Read the model definition and answer for the solid it produces. Units are mm, in the model's axes. Face numbers are marked on the shaded views. Round coordinates to 2 decimals unless told otherwise and drop trailing zeros. Order: outer loops, then holes, each group sorted by start corner. A loop starts at its lowest first (then second) coordinate and runs counter-clockwise, first axis right, second up. Notation, with made-up numbers: (67.25, -27.5) -> (87.25, -27.5) arc R10 cw to (87.25, -8.5) -> close; hole circle Ø9 at (-4.5, 15). An arc over 180 degrees is marked (long way). Answer as a JSON object with one key per item and string values. Group by question number.
Item 1: Given P1, Ø5, axis at x = 0, y = 0, coming from the +Z side; P2, Ø1, axis at y = -3, z = 7.5, coming from the -X side, each flat-ended and moving along its own axis, determine where each tip first touches the part or whether it passes through.
Item 2: The mould has two halves that part along X. Classify the marked faces 1, 2 and 3: pulls with the +X half, pulls with the -X half, needs draft (parallel to the pull), parting line crosses it, or undercut.
Item 3: Section A-A, the plane y = 0 is taken. Write down the section's boundary in (x, z).
Item 4: Section C-C, the plane x = 19.5 is taken. Write down the section's boundary in (y, z).
Item 5: Consider probe 1 along Y at (x, z) = (0, 2.5); probe 2 along X at (y, z) = (1.5, 4.25); probe 3 along X at (y, z) = (1, 4.5). Determine where each line is inside the solid, lowest interval first. Write a range as from..to.
Item 6: Section D-D, the plane y = -2.25 is taken. Write down the section's boundary in (x, z), plus the area to 3 significant figures.
Item 7: Section B-B, the plane z = 3.5 is taken. Write down the section's boundary in (x, y).
from build123d import *

# Parameters (mm, degrees)
SKETCH1_R           = 3
BOSS_EXTRUDE1_DEPTH = 10


with BuildPart() as part:
    # Sketch1 → Boss-Extrude1 (new body)
    with BuildSketch(Plane.XY):
        with BuildLine():
            Line((0, -6), (20, -6))
            ThreePointArc((20, -6), (26, 0), (20, 6))
            Line((20, 6), (0, 6))
            ThreePointArc((0, 6), (-6, 0), (0, -6))
        make_face()
        Circle(SKETCH1_R, mode=Mode.SUBTRACT)
        with Locations((20, 0)):
            Circle(SKETCH1_R, mode=Mode.SUBTRACT)
    extrude(amount=BOSS_EXTRUDE1_DEPTH)


solid = part.part
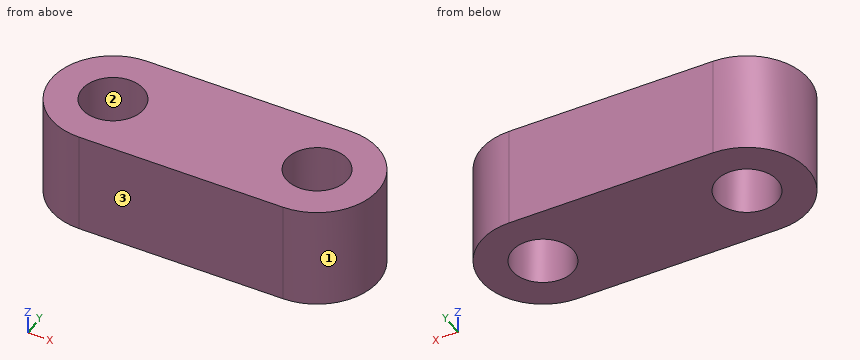
Values found:
{
 "1": {"P1": "through", "P2": "x = -5.45"},
 "2": {"face 1": "pulls with the +X half", "face 2": "undercut", "face 3": "needs draft"},
 "3": {"outline": "(-6, 0) -> (-3, 0) -> (-3, 10) -> (-6, 10) -> close; (3, 0) -> (17, 0) -> (17, 10) -> (3, 10) -> close; (23, 0) -> (26, 0) -> (26, 10) -> (23, 10) -> close"},
 "4": {"outline": "(-6, 0) -> (-2.96, 0) -> (-2.96, 10) -> (-6, 10) -> close; (2.96, 0) -> (6, 0) -> (6, 10) -> (2.96, 10) -> close"},
 "5": {"probe 1": "-6..-3, 3..6", "probe 2": "-5.81..-2.6, 2.6..17.4, 22.6..25.81", "probe 3": "-5.92..-2.83, 2.83..17.17, 22.83..25.92"},
 "6": {"outline": "(-5.56, 0) -> (-1.98, 0) -> (-1.98, 10) -> (-5.56, 10) -> close; (1.98, 0) -> (18.02, 0) -> (18.02, 10) -> (1.98, 10) -> close; (21.98, 0) -> (25.56, 0) -> (25.56, 10) -> (21.98, 10) -> close", "area": "232 mm2"},
 "7": {"outline": "(0, -6) -> (20, -6) arc R6 ccw to (20, 6) -> (0, 6) arc R6 ccw to start; hole circle Ø6 at (0, 0); hole circle Ø6 at (20, 0)"}
}
